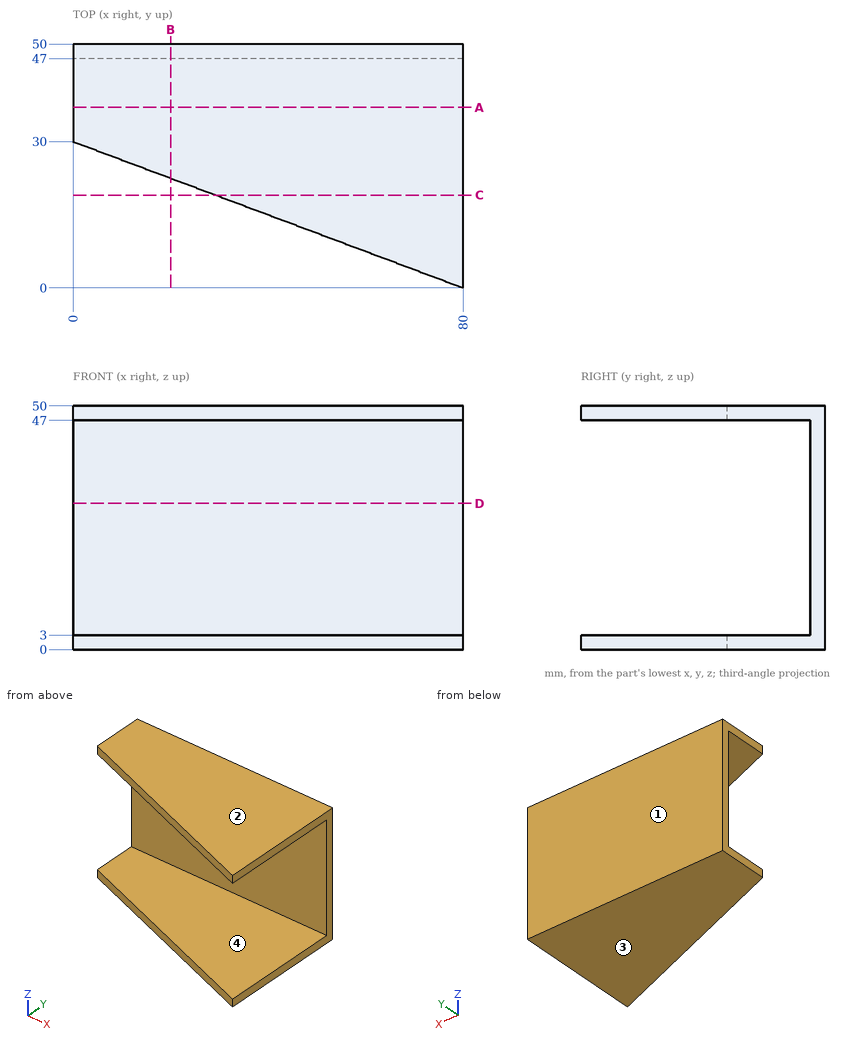
Drawing for the job (mm, zero at the part's lowest x, y, z). Round coordinates to 2 decimals unless told otherwise and drop trailing zeros. Write each loop counter-clockwise with the first axis right and the second up, starting at its lowest first coordinate (ties: lowest second). Pieces come first, ordered by that corner, then holes.
Item 1: Band-saw the part on D-D on z = 30. Write the cut outline in (x, y).
Filled in:
outline: (0, 47) - (80, 47) - (80, 50) - (0, 50) - close
Item 2: Band-saw the part on B-B on x = 20. Write the cut outline in (y, z), then the cut area to 3 significant figures.
Filled in:
outline: (22.5, 0) - (50, 0) - (50, 50) - (22.5, 50) - (22.5, 47) - (47, 47) - (47, 3) - (22.5, 3) - close
area: 297 mm2
Item 3: Band-saw the part on C-C on y = 19. Write the cut outline in (x, z).
Filled in:
outline: (29.33, 0) - (80, 0) - (80, 3) - (29.33, 3) - close; (29.33, 47) - (80, 47) - (80, 50) - (29.33, 50) - close
Item 4: Mould opens along Z. For the marked faces 1, 2, 3 and 4 say: released by +Z, released by -Z, zero draft, split by the parting line, or undercut.
Filled in:
face 1: zero draft
face 2: released by +Z
face 3: released by -Z
face 4: undercut
Item 5: Band-saw the part on A-A on y = 37. Write the cut outline in (x, z), then the cut area to 3 significant figures.
Filled in:
outline: (0, 0) - (80, 0) - (80, 3) - (0, 3) - close; (0, 47) - (80, 47) - (80, 50) - (0, 50) - close
area: 480 mm2
Item 6: Drop a flat-ended pin along its axis: pin 1 Ø6 at (x, z) = (66.5, 36) entering from -Y. Give the stop position or say it passes through.
Filled in:
pin 1: stops at y = 47
Item 7: Drill centre lines: L1, parallel to Z at x = 66.5, y = 27.5; L2, parallel to Y at x = 33, z = 29. Where is each one in solid material? Low to high.
Filled in:
L1: z = 0 to 3, 47 to 50
L2: y = 47 to 50
